Check sheet for the modelled part. Datum: model origin and axes. Units: mm. Give positions to 0.01 mm unless a question says otherwise; leave off trailing zeros. Write each loop counter-clockwise with the first axis right and the second up, starting at its lowest first coordinate (ties: lowest second). Pieces come first, ordered by that corner, then holes. Notation, with made-up numbers: M 76.5,76.25 L 99.5,76.25 A22 ccw 99.5,87.25 Z; hole C -10,35.5 d9. An arc over 180 degrees is marked long. Write item = value, one per line. Start each with the question number.
1) Scan lines: L1, parallel to X at y = 81.25, z = 0.5; L2, parallel to Z at x = -40, y = 81.5. Record each from-to range of solid material in increasing order.
2) Draft check along Z on faces 1 (the face through (42, 79, 1)), 2 (the face through (2.5, 83.1, 74)), 3 (the face through (-66.909, 83.042, 72.967)), 4 (the face through (38.05, 83.06, 63.08)). Enter one of: pulls with the +Z half, pulls with the -Z half, needs draft (parallel to the pull), parting line crosses it, or undercut.
3) Sectioned sample at C-C, the plane y = 82.25. Count the separate pieces of the cut face and the enclosed holes in it, then the cut area to 3 significant figures.
4) Sectioned sample at B-B, the plane x = 0. Record the cut outline in (y, z), then the cut area to 3 significant figures.
5) Gauge pin test, flat ends, axial feed: pin 1 (4 mm diameter, centred on x = -28.5, y = 80.5, fed in from -Z); pin 2 (2 mm diameter, centred on y = 83.5, z = 17.5, fed in from -X); pin 3 (4 mm diameter, centred on x = 36, y = 80, fed in from +Z). Record the tip position at first contact, or that the pin passes through.
6) Sectioned sample at A-A, the plane z = 0. Record the cut outline in (x, y), then the cut area to 3 significant figures.
from build123d import *

# Parameters (mm, degrees)
SKETCH_1_R      = 99
SKETCH_1_R_2    = 6.5
SKETCH_1_R_3    = 36.5
EXTRUDE_1_DEPTH = 8
CHAMFER_1_SIZE  = 1


with BuildPart() as part:
    # 草图1 → 凸台-拉伸1 (new body)
    with BuildSketch(Plane(origin=(0, 87, 0), x_dir=(1, 0, 0), z_dir=(0, 1, 0))):
        with Locations(Location((0, 0, 0), (0, 0, 90))):
            Circle(SKETCH_1_R)
        with Locations(Location((-80, 0, 0), (0, 0, 90))):
            Circle(SKETCH_1_R_2, mode=Mode.SUBTRACT)
        with Locations(Location((40, 69.282032303, 0), (0, 0, 90))):
            Circle(SKETCH_1_R_2, mode=Mode.SUBTRACT)
        with Locations(Location((-69.282032733, 40, 0), (0, 0, 90))):
            Circle(SKETCH_1_R_2, mode=Mode.SUBTRACT)
        with Locations(Location((-69.282032733, -39.999999255, 0), (0, 0, 90))):
            Circle(SKETCH_1_R_2, mode=Mode.SUBTRACT)
        with Locations(Location((0, 80, 0), (0, 0, 90))):
            Circle(SKETCH_1_R_2, mode=Mode.SUBTRACT)
        with Locations(Location((69.282032302, -39.999999255, 0), (0, 0, 90))):
            Circle(SKETCH_1_R_2, mode=Mode.SUBTRACT)
        with Locations(Location((-40, 69.282032303, 0), (0, 0, 90))):
            Circle(SKETCH_1_R_2, mode=Mode.SUBTRACT)
        with Locations(Location((0, -80, 0), (0, 0, 90))):
            Circle(SKETCH_1_R_2, mode=Mode.SUBTRACT)
        with Locations(Location((40, -69.282032303, 0), (0, 0, 90))):
            Circle(SKETCH_1_R_2, mode=Mode.SUBTRACT)
        with Locations(Location((69.282032302, 40, 0), (0, 0, 90))):
            Circle(SKETCH_1_R_2, mode=Mode.SUBTRACT)
        with Locations(Location((-40, -69.282032303, 0), (0, 0, 90))):
            Circle(SKETCH_1_R_2, mode=Mode.SUBTRACT)
        with Locations(Location((80, 0, 0), (0, 0, 90))):
            Circle(SKETCH_1_R_2, mode=Mode.SUBTRACT)
        with Locations(Location((0, 0, 0), (0, 0, 90))):
            Circle(SKETCH_1_R_3, mode=Mode.SUBTRACT)
    extrude(amount=-EXTRUDE_1_DEPTH)

    # 倒角1
    chamfer_1_edges = [part.edges().sort_by_distance(p)[0] for p in [
        (0, 87, 99),
        (0, 79, 99),
        (0, 79, 36.5),
        (0, 87, 36.5),
    ]]
    chamfer(chamfer_1_edges, length=CHAMFER_1_SIZE)


solid = part.part
Data:
q1.L1 = -99 to -86.48, -73.52 to -36.5, 36.5 to 73.52, 86.48 to 99
q1.L2 = -90.56 to -75.78, -62.78 to 62.78, 75.78 to 90.56
q2.face_1 = needs draft
q2.face_2 = undercut
q2.face_3 = parting line crosses it
q2.face_4 = undercut
q3.separate_pieces = 1
q3.enclosed_holes = 13
q3.area = 25,000 mm2
q4.outline = M 79,-98 L 80,-99 L 86,-99 L 87,-98 L 87,-86.5 L 79,-86.5 Z; M 79,-73.5 L 87,-73.5 L 87,-37.5 L 86,-36.5 L 80,-36.5 L 79,-37.5 Z; M 79,37.5 L 80,36.5 L 86,36.5 L 87,37.5 L 87,73.5 L 79,73.5 Z; M 79,86.5 L 87,86.5 L 87,98 L 86,99 L 80,99 L 79,98 Z
q4.area = 788 mm2
q5.pin_1 = -95.39
q5.pin_2 = -97.62
q5.pin_3 = 92.98
q6.outline = M -99,80 L -98,79 L -86.5,79 L -86.5,87 L -98,87 L -99,86 Z; M -73.5,79 L -37.5,79 L -36.5,80 L -36.5,86 L -37.5,87 L -73.5,87 Z; M 36.5,80 L 37.5,79 L 73.5,79 L 73.5,87 L 37.5,87 L 36.5,86 Z; M 86.5,79 L 98,79 L 99,80 L 99,86 L 98,87 L 86.5,87 Z
q6.area = 788 mm2
